```python
from build123d import *

# Parameters (mm, degrees)
SKETCH_1_W          = 50
SKETCH_1_H          = 25
EXTRUDE_1_DEPTH     = 30
SKETCH_2_R          = 2.75
CUT_EXTRUDE_1_DEPTH = 37


with BuildPart() as part:
    # 草图1 → 凸台-拉伸1 (new body)
    with BuildSketch(Plane.XY):
        with Locations((25, 12.5)):
            Rectangle(SKETCH_1_W, SKETCH_1_H)
    extrude(amount=EXTRUDE_1_DEPTH)

    # 草图2 → 切除-拉伸1 (cut)
    with BuildSketch(Plane.XY.offset(30)):
        with Locations((25, 7.5)):
            Circle(SKETCH_2_R)
    extrude(amount=-CUT_EXTRUDE_1_DEPTH, mode=Mode.SUBTRACT)


solid = part.part
```
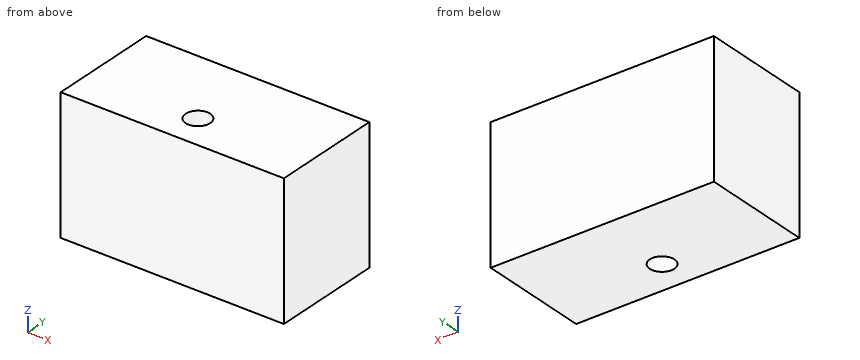
Part model, mm, in its own coordinate system. Give positions to 0.01 mm unless a question says otherwise; leave off trailing zeros. Order: outer loops, then holes, each group sorted by start corner. A loop starts at its lowest first (then second) coordinate and runs counter-clockwise, first axis right, second up. Notation, with made-up numbers: M 4.5,-15 L 26.5,-15 A20 cw 26.5,1 Z; hole C -27.75,6.5 d3. An arc over 180 degrees is marked long. Use a Markdown table: item, result. Add a question column.
(1) Saw through at A-A, the plane x = 25. Give the cut face in (y, z).
(2) Saw through at B-B, the plane y = 7.5. Give the cut face in (x, z), and give its area (4 significant figures).
(3) Drop a flat-ended pin along its axis: P1, Ø4.5, axis at x = 25, y = 7.5, coming from the +Z side. Give the stop position or say it passes through.
(4) Probe line 1 along Y through (x, z) = (25, 14); line 2 along X through (y, z) = (7.75, 20); line 3 along X through (y, z) = (8.5, 22.5). List the from-to ranges inside material, lowest first. Write a range as [from, to].
(5) Saw through at C-C, the plane z = 3. Give the cut face in (x, y).
Answer key:
| question | item | result |
|---|---|---|
| 1 | outline | M 0,0 L 4.75,0 L 4.75,30 L 0,30 Z; M 10.25,0 L 25,0 L 25,30 L 10.25,30 Z |
| 2 | outline | M 0,0 L 22.25,0 L 22.25,30 L 0,30 Z; M 27.75,0 L 50,0 L 50,30 L 27.75,30 Z |
| 2 | area | 1,335 mm^2 |
| 3 | P1 | through |
| 4 | line 1 | [0, 4.75], [10.25, 25] |
| 4 | line 2 | [0, 22.26], [27.74, 50] |
| 4 | line 3 | [0, 22.44], [27.56, 50] |
| 5 | outline | M 0,0 L 50,0 L 50,25 L 0,25 Z; hole C 25,7.5 d5.5 |
